Could you check a few things on this model? Use its own coordinates, in mm. A direction names the side the tool comes from. Round coordinates to 2 decimals unless told otherwise and drop trailing zeros. Loops run counter-clockwise (first coordinate to the right, second up) from the corner with the lowest first, then second, coordinate; pieces in that order, holes last. Notation, with made-up numbers: (-6, 26) -> (1, 26) arc R6 cw to (1, 35) -> close; hole circle Ø5 at (-23, -3). An arc over 180 degrees is marked (long way). Write each question's results on one line, items separated by ' | '. Start each with the question number.
1) Imagine slicing it at B-B, the plane x = -35. List the corners of the cut face in (y, z) for me, plus the area to 3 significant figures.
2) For P1, Ø9, axis at x = 34.5, y = 39, coming from the -Z side; P2, Ø6, axis at x = 17.5, z = -4.5, coming from the +Y side; P3, Ø2.5, axis at x = -33.5, y = 40.5, coming from the -Z side, each with a flat end and sliding along its axis, tell me the tip position at first contact or that it passes through.
3) Which directions (+Z, -Z, +X, -X, +Y, -Y) give clear straight access to the entire face, cutting with the end or side of a thin tool? Please do faces 1 (the flat face through (41, -1, 3)), 2 (the flat face through (10, 3, 4)).
4) Imagine slicing it at D-D, the plane y = 40. List the corners of the cut face in (x, z) for me.
5) We'd pull the mould along Y, two halves only. Please class faces 3 (the cylindrical face through (15.446, 3.604, -3.944)), 4 (the cylindrical face through (35.521, 43.966, 1.972)), 5 (the flat face through (-1, -50, 3)), 6 (the flat face through (-33, 38, 4)): pulls with the +Y half, pulls with the -Y half, needs draft (parallel to the pull), parting line crosses it, or undercut.
6) If I drill on probe 1 along Y at (x, z) = (-35, 1.8); probe 2 along Y at (x, z) = (35, 4.8); probe 3 along Y at (x, z) = (4, 4.55), over which ranges is the centre line in solid material (lowest first)?
7) Imagine slicing it at C-C, the plane y = 0. List the corners of the cut face in (x, z) for me.
8) Imagine slicing it at A-A, the plane x = 4. List the corners of the cut face in (y, z) for me.
from build123d import *

# Parameters (mm, degrees)
SKETCH_1_W           = 82
SKETCH_1_H           = 100
EXTRUDE_1_DEPTH      = 6
SKETCH_3_R           = 12
EXTRUDE_3_DEPTH      = 14
SKETCH_7_R           = 4
CUT_EXTRUDE_4_DEPTH  = 4
SKETCH_5_R           = 6.5
CUT_EXTRUDE_8_DEPTH  = 2
SKETCH_11_R          = 7.5
CUT_EXTRUDE_9_DEPTH  = 12
SKETCH_12_R          = 2.5
CUT_EXTRUDE_10_DEPTH = 6


with BuildPart() as part:
    # 草图1 → 凸台-拉伸1 (new body)
    with BuildSketch(Plane.XY):
        Rectangle(SKETCH_1_W, SKETCH_1_H)
    extrude(amount=EXTRUDE_1_DEPTH)

    # 草图3 → 凸台-拉伸3 (add)
    with BuildSketch(Plane.XY.offset(6)):
        with Locations((4, 0)):
            Circle(SKETCH_3_R)
    extrude(amount=-EXTRUDE_3_DEPTH)

    # 草图7 → 切除-拉伸4 (cut)
    with BuildSketch(Plane(origin=(0, 0, 0), x_dir=(-1, 0, 0), z_dir=(0, 0, -1))):
        with Locations((-35, 40)):
            Circle(SKETCH_7_R)
        with Locations(Location((-35, -40, 0), (0, 0, 180))):
            Circle(SKETCH_7_R)
        with Locations((35, -40)):
            Circle(SKETCH_7_R)
        with Locations(Location((35, 40, 0), (0, 0, 180))):
            Circle(SKETCH_7_R)
    extrude(amount=-CUT_EXTRUDE_4_DEPTH, mode=Mode.SUBTRACT)

    # 草图5 → 切除-拉伸8 (cut)
    with BuildSketch(Plane.XY.offset(6)):
        with Locations((4, 0)):
            Circle(SKETCH_5_R)
    extrude(amount=-CUT_EXTRUDE_8_DEPTH, mode=Mode.SUBTRACT)

    # 草图11 → 切除-拉伸9 (cut)
    with BuildSketch(Plane(origin=(0, 0, -8), x_dir=(-1, 0, 0), z_dir=(0, 0, -1))):
        with Locations((-4, 0)):
            Circle(SKETCH_11_R)
    extrude(amount=-CUT_EXTRUDE_9_DEPTH, mode=Mode.SUBTRACT)

    # 草图12 → 切除-拉伸10 (cut)
    with BuildSketch(Plane(origin=(0, 0, 0), x_dir=(-1, 0, 0), z_dir=(0, 0, -1))):
        with Locations((-35, -40)):
            Circle(SKETCH_12_R)
        with Locations((-35, 40)):
            Circle(SKETCH_12_R)
        with Locations((35, -40)):
            Circle(SKETCH_12_R)
        with Locations((35, 40)):
            Circle(SKETCH_12_R)
    extrude(amount=-CUT_EXTRUDE_10_DEPTH, mode=Mode.SUBTRACT)


solid = part.part
Checked values:
1) outline: (-50, 0) -> (-44, 0) -> (-44, 4) -> (-42.5, 4) -> (-42.5, 6) -> (-50, 6) -> close; (-37.5, 4) -> (-36, 4) -> (-36, 0) -> (36, 0) -> (36, 4) -> (37.5, 4) -> (37.5, 6) -> (-37.5, 6) -> close; (42.5, 4) -> (44, 4) -> (44, 0) -> (50, 0) -> (50, 6) -> (42.5, 6) -> close | area: 516 mm^2
2) P1: z = 0 | P2: y = 5.81 | P3: z = 4
3) face 1: +Z, -Z, +X, +Y, -Y | face 2: -Z
4) outline: (-41, 0) -> (-39, 0) -> (-39, 4) -> (-37.5, 4) -> (-37.5, 6) -> (-41, 6) -> close; (-32.5, 4) -> (-31, 4) -> (-31, 0) -> (31, 0) -> (31, 4) -> (32.5, 4) -> (32.5, 6) -> (-32.5, 6) -> close; (37.5, 4) -> (39, 4) -> (39, 0) -> (41, 0) -> (41, 6) -> (37.5, 6) -> close
5) face 3: parting line crosses it | face 4: undercut | face 5: pulls with the -Y half | face 6: undercut
6) probe 1: -50 to -44, -36 to 36, 44 to 50 | probe 2: -50 to -42.5, -37.5 to 37.5, 42.5 to 50 | probe 3: -50 to -6.5, 6.5 to 50
7) outline: (-41, 0) -> (-8, 0) -> (-8, -8) -> (-3.5, -8) -> (-3.5, 4) -> (-2.5, 4) -> (-2.5, 6) -> (-41, 6) -> close; (10.5, 4) -> (11.5, 4) -> (11.5, -8) -> (16, -8) -> (16, 0) -> (41, 0) -> (41, 6) -> (10.5, 6) -> close
8) outline: (-50, 0) -> (-12, 0) -> (-12, -8) -> (-7.5, -8) -> (-7.5, 4) -> (-6.5, 4) -> (-6.5, 6) -> (-50, 6) -> close; (6.5, 4) -> (7.5, 4) -> (7.5, -8) -> (12, -8) -> (12, 0) -> (50, 0) -> (50, 6) -> (6.5, 6) -> close
